Verification items for the finished model (mm, model axes). A direction names the side the tool comes from. Coordinates: 2 decimals unless noted, no trailing zeros. Order: outer loops, then holes, each group sorted by start corner. A loop starts at its lowest first (then second) coordinate and runs counter-clockwise, first axis right, second up. Notation, with made-up numbers: M 52.25,-38.5 L 65.25,-38.5 A26 ccw 65.25,-13.5 Z; hole C -26.5,51.25 d9. An arc over 180 degrees is marked long. Return JSON: item names as keys, results as strings.
```python
from build123d import *

# Parameters (mm, degrees)
SKETCH_1_W          = 180
SKETCH_1_H          = 150
EXTRUDE_1_DEPTH     = 6
CUT_EXTRUDE_1_REACH = 119.307
SKETCH_2_W          = 20
SKETCH_2_H          = 100


with BuildPart() as part:
    # 草图1 → 凸台-拉伸1 (new body)
    with BuildSketch(Plane.XY):
        Rectangle(SKETCH_1_W, SKETCH_1_H)
    extrude(amount=EXTRUDE_1_DEPTH)

    # 草图2 → 切除-拉伸1 (cut, up to next)
    with BuildSketch(Plane.XY.offset(6), mode=Mode.PRIVATE) as cut_extrude_1_sk1:
        with Locations((-45, -25)):
            Rectangle(SKETCH_2_W, SKETCH_2_H)
    cut_extrude_1_tool1 = extrude(cut_extrude_1_sk1.sketch, amount=-CUT_EXTRUDE_1_REACH, mode=Mode.PRIVATE) & part.part
    cut_extrude_1 = cut_extrude_1_tool1.solids().sort_by_distance((-45, -25, 6))[0]
    add(cut_extrude_1, mode=Mode.SUBTRACT)

    # 镜向1: 切除-拉伸1 across plane
    add(cut_extrude_1.mirror(Plane(origin=(0, 0, 0), x_dir=(0, 0, 1), z_dir=(1, 0, 0))), mode=Mode.SUBTRACT)


solid = part.part
```
Q1. Tool access check on faces 4 (the face through (45, 25, 3)), 5 (the face through (0, -75, 3)). Record the directions out of +Z, -Z, +X, -X, +Y, -Y that give a thin tool (end or side, any length) a straight path to the whole face; none if there is none.
Values:
{"face 4": "+Z, -Z, -Y", "face 5": "+Z, -Z, +X, -X, -Y"}
Q2. Cross-section at A-A, the plane y = -41. Record the boundary of the cut face in (x, z), and give its area (3 significant figures).
Values:
{"outline": "M -90,0 L -55,0 L -55,6 L -90,6 Z; M -35,0 L 35,0 L 35,6 L -35,6 Z; M 55,0 L 90,0 L 90,6 L 55,6 Z", "area": "840 mm^2"}
Q3. Cross-section at C-C, the plane x = -44.5. Record the boundary of the cut face in (y, z).
Values:
{"outline": "M 25,0 L 75,0 L 75,6 L 25,6 Z"}
Q4. Go/stop test with a flat-tipped pin: pin 1 (1.8 mm diameter, centred on x = -42.5, z = 2, fed in from -Y). Record where the tip stops, or that it passes through.
Values:
{"pin 1": "y = 25"}
Q5. Draft check along X on faces 1 (the face through (-90, -1, 3)), 2 (the face through (-55, -26, 3)), 3 (the face through (-1, 1, 6)). Enter one of: pulls with the +X half, pulls with the -X half, needs draft (parallel to the pull), parting line crosses it, or undercut.
Values:
{"face 1": "pulls with the -X half", "face 2": "undercut", "face 3": "needs draft"}
Q6. Cross-section at B-B, the plane z = 1.45. Record the boundary of the cut face in (x, y).
Values:
{"outline": "M -90,-75 L -55,-75 L -55,25 L -35,25 L -35,-75 L 35,-75 L 35,25 L 55,25 L 55,-75 L 90,-75 L 90,75 L -90,75 Z"}
Q7. Material ranges on line 1 along X through (y, z) = (-11.5, 2); line 2 along Y through (x, z) = (49, 1), recorded low to high.
Values:
{"line 1": "-90 to -55, -35 to 35, 55 to 90", "line 2": "25 to 75"}
